The model under review builds one solid part; all positions refer to its coordinate system, in mm. A direction names the side the tool comes from. Give positions to 0.01 mm unless a question says otherwise; leave off trailing zeros. Loops run counter-clockwise (first coordinate to the right, second up) from the corner with the lowest first, then second, coordinate; pieces in that order, holes last. Notation, with made-up numbers: M 39,-14.75 L 97,-14.75 A18 ccw 97,11.25 Z; hole C 72,5.5 d6. An arc over 180 degrees is marked long. One line per item, written item: value. Start each with the question number.
Q1. We need section A-A on z = 0. Write out the cut boundary in (x, y), plus the area to 3 significant figures.
Q2. To check wall thickness, follow line 1 along X through (y, z) = (-7.25, 0); line 2 along X through (y, z) = (0.5, 4); line 3 along X through (y, z) = (9.5, 5.75). State the ranges of each line that lie inside material, in increasing order. Write a range as from..to.
Q3. Mouldability with a two-part tool opening along Z and no side actions: class faces 3 (the face through (0.66, 5.916, -14.985)), 4 (the face through (4, 12, 0)), 5 (the face through (-4.9, -2.79, 1.79)) as released by +Z, released by -Z, zero draft, split by the parting line, or undercut.
Q4. We need section B-B on x = 8.5. Write out the cut boundary in (y, z).
Q5. We need section C-C on y = 4.5. Write out the cut boundary in (x, z), plus the area to 3 significant figures.
Q6. For faces 1 (the face through (-13.67, -8.87, 3.03)), 2 (the face through (7, -3, 1)), list the 3-axis set-ups (+Z, -Z, +X, -X, +Y, -Y) from which the entire face can be reached by the end or side of a thin tool; tool diameter is ignored.
Q7. We need section D-D on x = -2.25. Write out the cut boundary in (y, z).
Q8. For pin 1 (1 mm diameter, centred on x = 7.5, y = -9.5, fed in from -Z); pin 2 (2 mm diameter, centred on x = -8.5, y = -3.5, fed in from -Z); pin 3 (1.5 mm diameter, centred on y = 0, z = 3, fed in from +X), all flat-tipped, find the tip position at first contact; note any pin that passes through.
```python
from build123d import *

# Parameters (mm, degrees)
UPPER_BODY_PROFILE_30_R         = 15
UPPER_BODY_30X12_DEPTH          = 12
LOWER_BODY_PROFILE_28_R         = 14
LOWER_BODY_28X18_DEPTH          = 18
OFFSET_HOLES_PROFILE_3X_6_R     = 3
OFFSET_THROUGH_HOLES_3X_6_DEPTH = 44
CENTER_HOLE_PROFILE_6_R         = 3
CENTER_THROUGH_HOLE_6_DEPTH     = 44


with BuildPart() as part:
    # Upper Body Profile Ø30 → Upper Body Ø30x12 (new body)
    with BuildSketch(Plane(origin=(0, 0, 0), x_dir=(1, 0, 0), z_dir=(0, 1, 0))):
        with Locations(Location((0, 0, 0), (0, 0, 270))):
            Circle(UPPER_BODY_PROFILE_30_R)
    extrude(amount=UPPER_BODY_30X12_DEPTH)

    # Lower Body Profile Ø28 → Lower Body Ø28x18 (add)
    with BuildSketch(Plane.XZ):
        with Locations(Location((0, 0, 0), (0, 0, 270))):
            Circle(LOWER_BODY_PROFILE_28_R)
    extrude(amount=LOWER_BODY_28X18_DEPTH)

    # Offset Holes Profile 3xØ6 → Offset Through Holes 3xØ6 (cut)
    with BuildSketch(Plane(origin=(0, 12, 0), x_dir=(1, 0, 0), z_dir=(0, 1, 0))):
        with Locations(Location((0, 8, 0), (0, 0, 270))):
            Circle(OFFSET_HOLES_PROFILE_3X_6_R)
        with Locations(Location((6.92820323, -4, 0), (0, 0, 270))):
            Circle(OFFSET_HOLES_PROFILE_3X_6_R)
        with Locations(Location((-6.92820323, -4, 0), (0, 0, 270))):
            Circle(OFFSET_HOLES_PROFILE_3X_6_R)
    extrude(amount=-OFFSET_THROUGH_HOLES_3X_6_DEPTH, mode=Mode.SUBTRACT)

    # Center Hole Profile Ø6 → Center Through Hole Ø6 (cut)
    with BuildSketch(Plane(origin=(0, 12, 0), x_dir=(1, 0, 0), z_dir=(0, 1, 0))):
        with Locations(Location((0, 0, 0), (0, 0, 270))):
            Circle(CENTER_HOLE_PROFILE_6_R)
    extrude(amount=-CENTER_THROUGH_HOLE_6_DEPTH, mode=Mode.SUBTRACT)


solid = part.part
```
Solved:
1. outline: M -15,0 L -14,0 L -14,-18 L -3,-18 L -3,12 L -15,12 Z; M 3,-18 L 14,-18 L 14,0 L 15,0 L 15,12 L 3,12 Z
1. area: 684 mm2
2. line 1: -14..-3, 3..14
2. line 2: -14.46..-9.93, -3.93..3.93, 9.93..14.46
2. line 3: -13.85..-9.36, -4.49..4.49, 9.36..13.85
3. face 3: split by the parting line
3. face 4: zero draft
3. face 5: undercut
4. outline: M -18,-11.12 L 0,-11.12 L 0,-12.36 L 12,-12.36 L 12,1.44 L -18,1.44 Z; M -18,6.56 L 12,6.56 L 12,12.36 L 0,12.36 L 0,11.12 L -18,11.12 Z
5. outline: C 0,0 d30; hole C -6.93,4 d6; hole C 0,-8 d6; hole C 0,0 d6; hole C 6.93,4 d6
5. area: 594 mm2
6. face 1: -Y
6. face 2: +Y, -Y
7. outline: M -18,-13.82 L 0,-13.82 L 0,-14.83 L 12,-14.83 L 12,-9.98 L -18,-9.98 Z; M -18,-6.02 L 12,-6.02 L 12,-1.98 L -18,-1.98 Z; M -18,1.98 L 12,1.98 L 12,14.83 L 0,14.83 L 0,13.82 L -18,13.82 Z
8. pin 1: z = -12.12
8. pin 2: z = -11.82
8. pin 3: x = 14.83
